Part model, mm, in its own coordinate system. Round coordinates to 2 decimals unless told otherwise and drop trailing zeros. Write each loop counter-clockwise with the first axis right and the second up, starting at its lowest first coordinate (ties: lowest second). Pieces come first, ordered by that corner, then holes. Notation, with made-up numbers: M 53.25,28.25 L 99.25,28.25 A23 ccw 99.25,65.25 Z; hole C 73.25,23.25 d10. An arc over 180 degrees is marked long. Answer as a JSON object with one key per item and string values. Group by question number.
1. Drop flat-ended pins along their axis: pin 1 (5 mm diameter, centred on y = -13, z = 8, fed in from +X); pin 2 (8 mm diameter, centred on y = -10.5, z = 13, fed in from +X); pin 3 (6 mm diameter, centred on y = 0, z = 7.5, fed in from -X); pin 4 (4 mm diameter, centred on x = 10.5, y = -14, fed in from -Z). Give the stop position or say it passes through.
2. Drill centre lines: line 1 (Y direction, x = 0, z = 11); line 2 (X direction, y = -9, z = 2); line 3 (Y direction, x = 1.5, z = 2). Where is each one in solid material? Low to high. Write a range as from..to.
3. Band-saw the part on A-A, the plane x = 0. Write the cut outline in (y, z).
4. Two-plate mould, pull along Y, no slides. Class faces 1 (the face through (-2.17, -9.76, 7.4)), 2 (the face through (-0.2, -10.2, 0)), 3 (the face through (0, 18, 7)): +Y half, -Y half, draft (parallel to the pull), parting line (faces both ways), or undercut.
5. Band-saw the part on B-B, the plane z = 3.75. Write the cut outline in (x, y), plus the area to 3 significant figures.
from build123d import *

# Parameters (mm, degrees)
SKETCH1_R           = 10
BOSS_EXTRUDE1_DEPTH = 15


with BuildPart() as part:
    # Sketch1 → Boss-Extrude1 (new body)
    with BuildSketch(Plane.XY):
        Polygon((-20.784609691, 0), (-10.392304845, -18), (10.392304845, -18), (20.784609691, 0), (10.392304845, 18), (-10.392304845, 18), align=None)
        Circle(SKETCH1_R, mode=Mode.SUBTRACT)
    extrude(amount=BOSS_EXTRUDE1_DEPTH)

    # Sketch2 → Cut-Revolve1 (revolve, cut)
    with BuildSketch(Plane(origin=(0, 0, 0), x_dir=(1, 0, 0), z_dir=(0, 1, 0))):
        Polygon((13.784609691, 0.5), (25.784609691, -2.715390309), (25.784609691, 0.5), align=None)
        Polygon((25.784609691, -15.5), (25.784609691, -12.284609691), (13.784609691, -15.5), align=None)
    revolve(axis=Axis((0, 0, 15), (0, 0, -1)), mode=Mode.SUBTRACT)


solid = part.part
Worked answers:
{
 "1": {"pin 1": "stops at x = 14.72", "pin 2": "stops at x = 17.03", "pin 3": "stops at x = -20.78", "pin 4": "stops at z = 0"},
 "2": {"line 1": "y = -18..-10, 10..18", "line 2": "x = -15.59..-4.36, 4.36..15.59", "line 3": "y = -18..-9.89, 9.89..18"},
 "3": {"outline": "M -18,0.63 L -15.65,0 L -10,0 L -10,15 L -15.65,15 L -18,14.37 Z; M 10,0 L 15.65,0 L 18,0.63 L 18,14.37 L 15.65,15 L 10,15 Z"},
 "4": {"face 1": "undercut", "face 2": "draft", "face 3": "+Y half"},
 "5": {"outline": "M -20.78,0 L -10.39,-18 L 10.39,-18 L 20.78,0 L 10.39,18 L -10.39,18 Z; hole C 0,0 d20", "area": "808 mm^2"}
}
